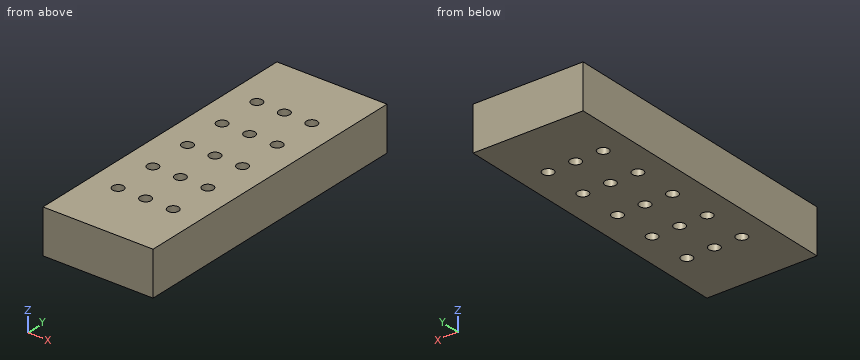
from build123d import *

# Parameters (mm, degrees)
SKETCH_1_W               = 10
SKETCH_1_H               = 27
EXTRUDE_1_DEPTH          = 4
CUT_EXTRUDE_1_REACH      = 16.942
SKETCH_2_R               = 0.5
PATTERN_LINEAR_2_COUNT   = 3
PATTERN_LINEAR_2_PITCH   = 4
MIRROR_1_COPY_1_REACH    = 16.942
MIRROR_1_COPY_1_SKETCH_R = 0.5
MIRROR_1_COPY_2_REACH    = 16.942
MIRROR_1_COPY_2_SKETCH_R = 0.5


with BuildPart() as part:
    # Sketch 1 → Extrude 1 (new body)
    with BuildSketch(Plane.XY):
        Rectangle(SKETCH_1_W, SKETCH_1_H)
    extrude(amount=EXTRUDE_1_DEPTH)

    # Sketch 2 → Cut-Extrude 1 (cut, up to next)
    with BuildSketch(Plane.XY.offset(4), mode=Mode.PRIVATE) as cut_extrude_1_sk1:
        Circle(SKETCH_2_R)
    cut_extrude_1_tool1 = extrude(cut_extrude_1_sk1.sketch, amount=-CUT_EXTRUDE_1_REACH, mode=Mode.PRIVATE) & part.part
    # Sketch 2 → Cut-Extrude 1 (cut, up to next)
    with BuildSketch(Plane.XY.offset(4), mode=Mode.PRIVATE) as cut_extrude_1_sk2:
        with Locations((-2.5, 0)):
            Circle(SKETCH_2_R)
    cut_extrude_1_tool2 = extrude(cut_extrude_1_sk2.sketch, amount=-CUT_EXTRUDE_1_REACH, mode=Mode.PRIVATE) & part.part
    # Sketch 2 → Cut-Extrude 1 (cut, up to next)
    with BuildSketch(Plane.XY.offset(4), mode=Mode.PRIVATE) as cut_extrude_1_sk3:
        with Locations((2.5, 0)):
            Circle(SKETCH_2_R)
    cut_extrude_1_tool3 = extrude(cut_extrude_1_sk3.sketch, amount=-CUT_EXTRUDE_1_REACH, mode=Mode.PRIVATE) & part.part
    cut_extrude_1_1 = cut_extrude_1_tool1.solids().sort_by_distance((0, 0, 4))[0]
    add(cut_extrude_1_1, mode=Mode.SUBTRACT)
    cut_extrude_1_2 = cut_extrude_1_tool2.solids().sort_by_distance((-2.5, 0, 4))[0]
    add(cut_extrude_1_2, mode=Mode.SUBTRACT)
    cut_extrude_1_3 = cut_extrude_1_tool3.solids().sort_by_distance((2.5, 0, 4))[0]
    add(cut_extrude_1_3, mode=Mode.SUBTRACT)
    cut_extrude_1 = cut_extrude_1_1 + cut_extrude_1_2 + cut_extrude_1_3  # Cut-Extrude 1 as one shape, for the pattern or mirror that repeats it

    # Pattern Linear 2: Cut-Extrude 1 ×3
    with Locations(*[(0, -i * PATTERN_LINEAR_2_PITCH, 0) for i in range(1, PATTERN_LINEAR_2_COUNT)]):
        add(cut_extrude_1, mode=Mode.SUBTRACT)

    # Mirror 1 copy 1 sketch → Mirror 1 copy 1 (cut, up to next)
    with BuildSketch(Plane(origin=(0, 4, 4), x_dir=(1, 0, 0), z_dir=(0, 0, 1)), mode=Mode.PRIVATE) as mirror_1_copy_1_sk1:
        Circle(MIRROR_1_COPY_1_SKETCH_R)
    mirror_1_copy_1_tool1 = extrude(mirror_1_copy_1_sk1.sketch, amount=-MIRROR_1_COPY_1_REACH, mode=Mode.PRIVATE) & part.part
    # Mirror 1 copy 1 sketch → Mirror 1 copy 1 (cut, up to next)
    with BuildSketch(Plane(origin=(0, 4, 4), x_dir=(1, 0, 0), z_dir=(0, 0, 1)), mode=Mode.PRIVATE) as mirror_1_copy_1_sk2:
        with Locations((-2.5, 0)):
            Circle(MIRROR_1_COPY_1_SKETCH_R)
    mirror_1_copy_1_tool2 = extrude(mirror_1_copy_1_sk2.sketch, amount=-MIRROR_1_COPY_1_REACH, mode=Mode.PRIVATE) & part.part
    # Mirror 1 copy 1 sketch → Mirror 1 copy 1 (cut, up to next)
    with BuildSketch(Plane(origin=(0, 4, 4), x_dir=(1, 0, 0), z_dir=(0, 0, 1)), mode=Mode.PRIVATE) as mirror_1_copy_1_sk3:
        with Locations((2.5, 0)):
            Circle(MIRROR_1_COPY_1_SKETCH_R)
    mirror_1_copy_1_tool3 = extrude(mirror_1_copy_1_sk3.sketch, amount=-MIRROR_1_COPY_1_REACH, mode=Mode.PRIVATE) & part.part
    add(mirror_1_copy_1_tool1.solids().sort_by_distance((0, 4, 4))[0], mode=Mode.SUBTRACT)
    add(mirror_1_copy_1_tool2.solids().sort_by_distance((-2.5, 4, 4))[0], mode=Mode.SUBTRACT)
    add(mirror_1_copy_1_tool3.solids().sort_by_distance((2.5, 4, 4))[0], mode=Mode.SUBTRACT)

    # Mirror 1 copy 2 sketch → Mirror 1 copy 2 (cut, up to next)
    with BuildSketch(Plane(origin=(0, 8, 4), x_dir=(1, 0, 0), z_dir=(0, 0, 1)), mode=Mode.PRIVATE) as mirror_1_copy_2_sk1:
        Circle(MIRROR_1_COPY_2_SKETCH_R)
    mirror_1_copy_2_tool1 = extrude(mirror_1_copy_2_sk1.sketch, amount=-MIRROR_1_COPY_2_REACH, mode=Mode.PRIVATE) & part.part
    # Mirror 1 copy 2 sketch → Mirror 1 copy 2 (cut, up to next)
    with BuildSketch(Plane(origin=(0, 8, 4), x_dir=(1, 0, 0), z_dir=(0, 0, 1)), mode=Mode.PRIVATE) as mirror_1_copy_2_sk2:
        with Locations((-2.5, 0)):
            Circle(MIRROR_1_COPY_2_SKETCH_R)
    mirror_1_copy_2_tool2 = extrude(mirror_1_copy_2_sk2.sketch, amount=-MIRROR_1_COPY_2_REACH, mode=Mode.PRIVATE) & part.part
    # Mirror 1 copy 2 sketch → Mirror 1 copy 2 (cut, up to next)
    with BuildSketch(Plane(origin=(0, 8, 4), x_dir=(1, 0, 0), z_dir=(0, 0, 1)), mode=Mode.PRIVATE) as mirror_1_copy_2_sk3:
        with Locations((2.5, 0)):
            Circle(MIRROR_1_COPY_2_SKETCH_R)
    mirror_1_copy_2_tool3 = extrude(mirror_1_copy_2_sk3.sketch, amount=-MIRROR_1_COPY_2_REACH, mode=Mode.PRIVATE) & part.part
    add(mirror_1_copy_2_tool1.solids().sort_by_distance((0, 8, 4))[0], mode=Mode.SUBTRACT)
    add(mirror_1_copy_2_tool2.solids().sort_by_distance((-2.5, 8, 4))[0], mode=Mode.SUBTRACT)
    add(mirror_1_copy_2_tool3.solids().sort_by_distance((2.5, 8, 4))[0], mode=Mode.SUBTRACT)


solid = part.part
Could you check a few things on this model? Use its own coordinates, in mm. Give positions to 0.01 mm unless a question says otherwise; leave off trailing zeros. Write each loop counter-clockwise with the first axis right and the second up, starting at its lowest first coordinate (ties: lowest second). Pieces come first, ordered by that corner, then holes. Notation, with made-up numbers: (55, -1.5) - (108, -1.5) arc R29 ccw to (108, 24.5) - close; hole circle Ø1 at (16.25, 70). An arc over 180 degrees is marked (long way). Use CSV: the item, a comma, the result in double quotes. Start each with the question number.
Item 1: I want a section at C-C, the plane z = 3.6. Give the number of separate pieces and of enclosed holes in the cut face, then the cut area to 3 significant figures.
Item 2: I want a section at B-B, the plane y = 4. Please give me the cut outline in (x, z), then the cut area to 3 significant figures.
Item 3: If I drill on line 1 along Y through (x, z) = (-2.5, 1.1); line 2 along Y through (x, z) = (-2.75, 0.2), over which ranges is the centre line in solid material (lowest first)?
Item 4: I want a section at A-A, the plane x = -2.5. Please give me the cut outline in (y, z), then the cut area to 3 significant figures.
Item 5: I want a section at D-D, the plane x = 0.25. Please give me the cut outline in (y, z).
Findings:
1,separate pieces,"1"
1,enclosed holes,"15"
1,area,"258 mm2"
2,outline,"(-5, 0) - (-3, 0) - (-3, 4) - (-5, 4) - close; (-2, 0) - (-0.5, 0) - (-0.5, 4) - (-2, 4) - close; (0.5, 0) - (2, 0) - (2, 4) - (0.5, 4) - close; (3, 0) - (5, 0) - (5, 4) - (3, 4) - close"
2,area,"28.0 mm2"
3,line 1,"y = -13.5 to -8.5, -7.5 to -4.5, -3.5 to -0.5, 0.5 to 3.5, 4.5 to 7.5, 8.5 to 13.5"
3,line 2,"y = -13.5 to -8.43, -7.57 to -4.43, -3.57 to -0.43, 0.43 to 3.57, 4.43 to 7.57, 8.43 to 13.5"
4,outline,"(-13.5, 0) - (-8.5, 0) - (-8.5, 4) - (-13.5, 4) - close; (-7.5, 0) - (-4.5, 0) - (-4.5, 4) - (-7.5, 4) - close; (-3.5, 0) - (-0.5, 0) - (-0.5, 4) - (-3.5, 4) - close; (0.5, 0) - (3.5, 0) - (3.5, 4) - (0.5, 4) - close; (4.5, 0) - (7.5, 0) - (7.5, 4) - (4.5, 4) - close; (8.5, 0) - (13.5, 0) - (13.5, 4) - (8.5, 4) - close"
4,area,"88.0 mm2"
5,outline,"(-13.5, 0) - (-8.43, 0) - (-8.43, 4) - (-13.5, 4) - close; (-7.57, 0) - (-4.43, 0) - (-4.43, 4) - (-7.57, 4) - close; (-3.57, 0) - (-0.43, 0) - (-0.43, 4) - (-3.57, 4) - close; (0.43, 0) - (3.57, 0) - (3.57, 4) - (0.43, 4) - close; (4.43, 0) - (7.57, 0) - (7.57, 4) - (4.43, 4) - close; (8.43, 0) - (13.5, 0) - (13.5, 4) - (8.43, 4) - close"
